Print and shaded views of the part. All mm, measured from the part's lowest x, y and z. A direction names the side the tool comes from. Round coordinates to 2 decimals unless told otherwise and drop trailing zeros. Write each loop counter-clockwise with the first axis right and the second up, starting at its lowest first coordinate (ties: lowest second). Pieces come first, ordered by that corner, then holes. Notation, with made-up numbers: (12.25, 73) - (66.25, 73) arc R24 cw to (66.25, 112) - close; hole circle Ø11 at (-3.75, 53). An arc over 180 degrees is marked (long way). Put each result on its own line as item: value. Start each with the question number.
Item 1: Pin check, flat tips, straight feed: pin 1 Ø12 at (x, y) = (43.5, 36.5) entering from +Z; pin 2 Ø8 at (x, y) = (11.5, 92) entering from -Z; pin 3 Ø12.5 at (y, z) = (142.5, 72.5) entering from +X. Stop position of each tip, or through.
Item 2: Cut at D-D (z = 62). Give the cut face in (x, y).
Item 3: Cut at C-C (x = 38). Give the cut face in (y, z).
Item 4: Cut at A-A (z = 42.5). Give the cut face in (x, y), and give its area (3 significant figures).
Item 5: Mould opens along Y. For the marked faces 4, 5, 6 and 7 say: released by +Y, released by -Y, zero draft, split by the parting line, or undercut.
Item 6: Cut at B-B (y = 136.5). Give the cut face in (x, z).
Item 7: 3-axis set-ups, long thin cutter, end or side, ignore diameter. For the marked faces 1, 2 and 3: which of +Z, -Z, +X, -X, +Y, -Y reach the whole face in a straight line?
Item 8: Drill centre lines: line 1 (Y direction, x = 37.5, z = 42); line 2 (X direction, y = 120, z = 52); line 3 (Y direction, x = 38, z = 82). Where is each one in solid material? Low to high. Write a range as from..to.
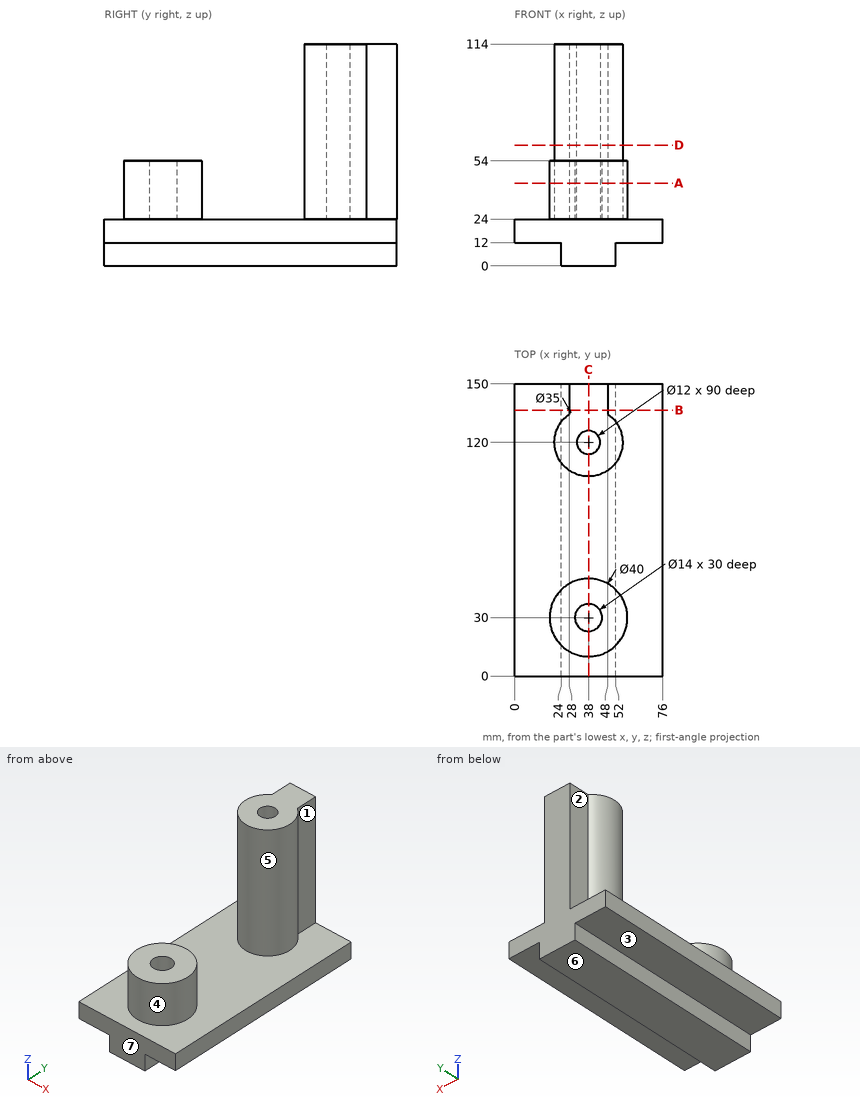
Output values:
1. pin 1: z = 54
1. pin 2: z = 12
1. pin 3: x = 48
2. outline: (28, 134.36) arc R17.5 ccw (long way) to (48, 134.36) - (48, 150) - (28, 150) - close; hole circle Ø12 at (38, 120)
3. outline: (0, 0) - (150, 0) - (150, 114) - (126, 114) - (126, 24) - (114, 24) - (114, 114) - (102.5, 114) - (102.5, 24) - (50, 24) - (50, 54) - (37, 54) - (37, 24) - (23, 24) - (23, 54) - (10, 54) - (10, 24) - (0, 24) - close
4. outline: circle Ø40 at (38, 30); (28, 134.36) arc R17.5 ccw (long way) to (48, 134.36) - (48, 150) - (28, 150) - close; hole circle Ø14 at (38, 30); hole circle Ø12 at (38, 120)
4. area: 2,220 mm2
5. face 4: undercut
5. face 5: undercut
5. face 6: zero draft
5. face 7: released by -Y
6. outline: (0, 12) - (24, 12) - (24, 0) - (52, 0) - (52, 12) - (76, 12) - (76, 24) - (48, 24) - (48, 114) - (28, 114) - (28, 24) - (0, 24) - close
7. face 1: +Z, +X, +Y
7. face 2: +Z, -X, +Y
7. face 3: -Z, -X, +Y, -Y
8. line 1: 10.01..23.02, 36.98..49.99, 102.51..114.02, 125.98..150
8. line 2: 20.5..32, 44..55.5
8. line 3: 102.5..114, 126..150
